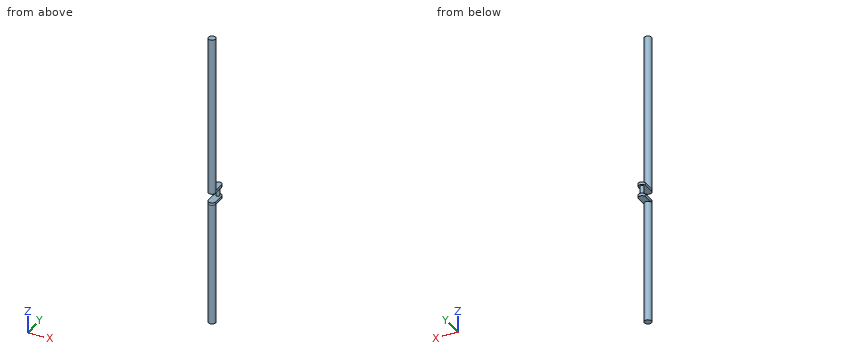
```python
from build123d import *

# Parameters (mm, degrees)
SKETCH1_R               = 10
BOSS_EXTRUDE1_DEPTH     = 362
CUT_EXTRUDE1_DEPTH      = 363.276137773
CUT_EXTRUDE1_DEPTH_BACK = 363.276137773
SKETCH2_W               = 145.080809864
SKETCH2_H               = 40
BOSS_EXTRUDE2_DEPTH     = 20
CUT_EXTRUDE2_DEPTH      = 365.751970522
CUT_EXTRUDE2_DEPTH_BACK = 365.751970522
SKETCH4_W               = 25
SKETCH4_H               = 210.962257982
SKETCH5_R               = 5
BOSS_EXTRUDE3_DEPTH     = 12.5
SKETCH6_R               = 10
BOSS_EXTRUDE4_DEPTH     = 95.2


with BuildPart() as part:
    # Sketch1 → Boss-Extrude1 (new, symmetric)
    with BuildSketch(Plane.XY):
        Circle(SKETCH1_R)
    extrude(amount=BOSS_EXTRUDE1_DEPTH, both=True)

    # Sketch2 → Cut-Extrude1 (cut, two sides: drawn at the far end of the back side and taken through both)
    with BuildSketch(Plane(origin=(0, 0, 0), x_dir=(1, 0, 0), z_dir=(0, 1, 0)).offset(-CUT_EXTRUDE1_DEPTH_BACK)):
        Rectangle(SKETCH2_W, SKETCH2_H)
    extrude(amount=CUT_EXTRUDE1_DEPTH + CUT_EXTRUDE1_DEPTH_BACK, mode=Mode.SUBTRACT)


with BuildPart() as cut_extrude1_piece_1:
    # of the separate pieces the step leaves, piece 1, a body of its own (cut_extrude1_pieces)
    add(part.part.solids().sort_by_distance((10, 0, -362))[0])



with BuildPart() as cut_extrude1_piece_2:
    # of the separate pieces the step leaves, piece 2, a body of its own (cut_extrude1_pieces)
    add(part.part.solids().sort_by_distance((10, 0, 20))[0])


with BuildPart() as cut_extrude1_piece_1_1:
    add(cut_extrude1_piece_1.part)

    add(cut_extrude1_piece_2.part)  # Boss-Extrude2 merges Cut-Extrude1 piece 2
    # Sketch3 → Boss-Extrude2 (add, symmetric)
    with BuildSketch(Plane.XY):
        with BuildLine():
            Line((-10, 0), (-10, 30))
            ThreePointArc((-10, 30), (0, 40), (10, 30))
            Line((10, 30), (10, 0))
            ThreePointArc((10, 0), (0, -10), (-10, 0))
        make_face()
    extrude(amount=BOSS_EXTRUDE2_DEPTH, both=True)

    # Sketch4 → Cut-Extrude2 (cut, two sides: drawn at the far end of the back side and taken through both)
    with BuildSketch(Plane(origin=(10, 0, 0), x_dir=(0, 0, -1), z_dir=(1, 0, 0)).offset(-CUT_EXTRUDE2_DEPTH_BACK)):
        Rectangle(SKETCH4_W, SKETCH4_H)
    extrude(amount=CUT_EXTRUDE2_DEPTH + CUT_EXTRUDE2_DEPTH_BACK, mode=Mode.SUBTRACT)


with BuildPart() as cut_extrude2_piece_1:
    # of the separate pieces the step leaves, piece 1, a body of its own (cut_extrude2_pieces)
    add(cut_extrude1_piece_1_1.part.solids().sort_by_distance((10, 0, 20))[0])



with BuildPart() as cut_extrude2_piece_2:
    # of the separate pieces the step leaves, piece 2, a body of its own (cut_extrude2_pieces)
    add(cut_extrude1_piece_1_1.part.solids().sort_by_distance((10, 0, -20))[0])


with BuildPart() as cut_extrude2_piece_1_1:
    add(cut_extrude2_piece_1.part)

    add(cut_extrude2_piece_2.part)  # Boss-Extrude3 merges Cut-Extrude2 piece 2
    # Sketch5 → Boss-Extrude3 (add, symmetric)
    with BuildSketch(Plane.XY):
        with Locations(Location((0, 30, 0), (0, 0, 180))):
            Circle(SKETCH5_R)
    extrude(amount=BOSS_EXTRUDE3_DEPTH, both=True)

    # Sketch6 → Boss-Extrude4 (add)
    with BuildSketch(Plane.XY.offset(362)):
        Circle(SKETCH6_R)
    extrude(amount=BOSS_EXTRUDE4_DEPTH)


solid = cut_extrude2_piece_1_1.part
```
Work out the finished part from the listing and answer in its coordinate system (mm). Give positions to 0.01 mm unless a question says otherwise; leave off trailing zeros. Loops run counter-clockwise (first coordinate to the right, second up) from the corner with the lowest first, then second, coordinate; pieces in that order, holes last. Notation, with made-up numbers: M -16.75,79.25 L 9.25,79.25 A36 cw 9.25,114.25 Z; hole C 78.25,57 d4. An arc over 180 degrees is marked long. One line per item, written item: value. Start each with the question number.
1. Each of these flat-tipped pins is pushed along its axis until it touches: P1, Ø10, axis at x = -2.5, y = 17, coming from the +Z side; P2, Ø10, axis at x = -0.5, z = -165, coming from the +Y side; P3, Ø8, axis at x = 7, z = -218.5, coming from the +Y side. Where does it stop, or does it pass through?
2. Find the intervals of material crossed by probe 1 along Z at (x, y) = (-5.25, 20); probe 2 along Z at (x, y) = (1.25, 2); probe 3 along Z at (x, y) = (-3, 29.5), in increasing order.
3. Find section A-A (x = 0). Give the vertices of the cut face in (y, z), and give its area (3 significant figures).
4. Find section B-B (z = 396). Give the vertices of the cut face in (x, y), and give its area (3 significant figures).
Reported:
1. P1: stops at z = 20
1. P2: stops at y = 10
1. P3: stops at y = 9.54
2. probe 1: z = -20 to -12.5, 12.5 to 20
2. probe 2: z = -362 to -12.5, 12.5 to 457.2
2. probe 3: z = -20 to 20
3. outline: M -10,-362 L 10,-362 L 10,-20 L 40,-20 L 40,-12.5 L 35,-12.5 L 35,12.5 L 40,12.5 L 40,20 L 10,20 L 10,457.2 L -10,457.2 L -10,12.5 L 25,12.5 L 25,-12.5 L -10,-12.5 Z
3. area: 16,600 mm²
4. outline: C 0,0 d20
4. area: 314 mm²
